For this review, take the finished solid that the model builds, in its own axes (mm). Round coordinates to 2 decimals unless told otherwise and drop trailing zeros. Write each loop counter-clockwise with the first axis right and the second up, starting at its lowest first coordinate (ties: lowest second). Pieces come first, ordered by that corner, then holes. Notation, with made-up numbers: (49.25, -28.75) -> (84.25, -28.75) arc R28 cw to (84.25, -7.75) -> close; hole circle Ø1 at (81.5, -30). An arc over 180 degrees is marked (long way). Answer as CSV lines item,"result". Start each with the question number.
Item 1: Mouldability with a two-part tool opening along X and no side actions: class faces 1 (the cylindrical face through (117.385, 20.751, 6.084)), 2 (the flat face through (-125, 0, 6)), 3 (the flat face through (-2, -35, 6)) as +X half, -X half, draft (parallel to the pull), parting line (faces both ways), or undercut.
Item 2: Wall thickness on probe 1 along Y at (x, z) = (100, 8); probe 2 along X at (y, z) = (19.5, 4.5); probe 3 along Y at (x, z) = (-46, 10): over which ranges is each line inside the solid? List them lowest first. Write a range as from..to.
Item 3: For pin 1 Ø8 at (x, y) = (-115, -20) entering from +Z; pin 2 Ø6.5 at (x, y) = (-100, -25) entering from -Z, all flat-tipped, find the tip position at first contact; note any pin that passes through.
Item 4: Take a section at B-B on z = 5.75. Count the separate pieces of the cut face and the enclosed holes in it, then the cut area to 3 significant figures.
Item 5: Take a section at A-A on x = 100. Give the boundary of the cut face in (y, z).
```python
from build123d import *

# Parameters (mm, degrees)
SKETCH_1_W            = 250
SKETCH_1_H            = 70
EXTRUDE_1_DEPTH       = 12
CHAMFER_1_SIZE        = 3
HOLE_WIZARD_7_0_7_1_D = 7
HOLE_WIZARD_M6_1_D    = 5
HOLE_WIZARD_7_0_7_2_D = 7


with BuildPart() as part:
    # 草图1 → 凸台-拉伸1 (new body)
    with BuildSketch(Plane.XY):
        Rectangle(SKETCH_1_W, SKETCH_1_H)
    extrude(amount=EXTRUDE_1_DEPTH)

    # 倒角1
    chamfer_1_edges = [part.edges().sort_by_distance(p)[0] for p in [
        (125, -35, 6),
        (-125, -35, 6),
        (-125, 35, 6),
        (125, 35, 6),
    ]]
    chamfer(chamfer_1_edges, length=CHAMFER_1_SIZE)

    # Ø7.0 (7) 直径孔1 (through all)
    with Locations(Plane(origin=(0, 0, 0), x_dir=(-1, 0, 0), z_dir=(0, 0, -1))):
        with Locations((100, -25), (100, 25), (-100, 25), (-100, -25)):
            Hole(HOLE_WIZARD_7_0_7_1_D / 2)

    # M6 螺纹孔1 (through all)
    with Locations(Plane(origin=(0, 0, 0), x_dir=(-1, 0, 0), z_dir=(0, 0, -1))):
        with Locations((115, -20), (115, 20), (-115, 20), (-115, -20)):
            Hole(HOLE_WIZARD_M6_1_D / 2)

    # Ø7.0 (7) 直径孔2 (through all)
    with Locations(Plane(origin=(0, 0, 0), x_dir=(-1, 0, 0), z_dir=(0, 0, -1))):
        with Locations((46, 27.5), (46, -27.5), (-46, 27.5), (-46, -27.5)):
            Hole(HOLE_WIZARD_7_0_7_2_D / 2)


solid = part.part
```
Output values:
1,face 1,"undercut"
1,face 2,"-X half"
1,face 3,"draft"
2,probe 1,"y = -35..-28.5, -21.5..21.5, 28.5..35"
2,probe 2,"x = -125..-117.45, -112.55..112.55, 117.45..125"
2,probe 3,"y = -35..-31, -24..24, 31..35"
3,pin 1,"stops at z = 12"
3,pin 2,"passes through"
4,separate pieces,"1"
4,enclosed holes,"12"
4,area,"17,100 mm^2"
5,outline,"(-35, 0) -> (-28.5, 0) -> (-28.5, 12) -> (-35, 12) -> close; (-21.5, 0) -> (21.5, 0) -> (21.5, 12) -> (-21.5, 12) -> close; (28.5, 0) -> (35, 0) -> (35, 12) -> (28.5, 12) -> close"
